CAD build for the part. Positions are in the model's coordinates, mm. A direction names the side the tool comes from. Coordinates: 2 decimals unless noted, no trailing zeros. Write each loop counter-clockwise with the first axis right and the second up, starting at its lowest first coordinate (ties: lowest second). Pieces come first, ordered by that corner, then holes. Notation, with made-up numbers: (49, 49) - (72, 49) arc R28 ccw to (72, 71) - close; hole circle Ø2 at (57.5, 76.25). An arc over 180 degrees is marked (long way). One line per question, with ' | ' between items. Start each with the question number.
1. Band-saw the part on A-A, the plane x = 0. Write the cut outline in (y, z), then the cut area to 4 significant figures.
2. Band-saw the part on C-C, the plane y = 19.5. Write the cut outline in (x, z).
3. Which spindle directions (+Z, -Z, +X, -X, +Y, -Y) get a long thin tool onto all of the face, cutting with end or side? Do faces 1 (the cylindrical face through (0.33, 29.684, -7.493)), 2 (the flat face through (-5, 25, 2)). Say none if no direction does.
4. Flat gauge pins, fed straight in: P1, Ø5, axis at y = -8, z = 0.5, coming from the -X side; P2, Ø4, axis at x = 0, y = 20, coming from the -Z side; P3, Ø3, axis at x = 1.5, y = -9.5, coming from the +Z side. Where does each tip first touch, or does it go through?
5. Band-saw the part on B-B, the plane z = 0. Write the cut outline in (x, y), then the cut area to 4 significant figures.
6. Probe line 1 (X direction, y = -16.5, z = 0.25); line 2 (Y direction, x = 6.25, z = -2); line 3 (X direction, y = 32.5, z = -1.25). List the from-to ranges inside material, lowest first.
from build123d import *

# Parameters (mm, degrees)
SKETCH_1_R      = 5
EXTRUDE_1_DEPTH = 25
SKETCH_2_R      = 7.5
EXTRUDE_2_DEPTH = 10
CHAMFER_1_SIZE  = 0.5


with BuildPart() as part:
    # 草图1 → 凸台-拉伸1 (new, symmetric)
    with BuildSketch(Plane(origin=(0, 0, 0), x_dir=(1, 0, 0), z_dir=(0, 1, 0))):
        with Locations(Location((0, 0, 0), (0, 0, 270))):
            Circle(SKETCH_1_R)
    extrude(amount=EXTRUDE_1_DEPTH, both=True)

    # 草图2 → 凸台-拉伸2 (add)
    with BuildSketch(Plane(origin=(0, 25, 0), x_dir=(1, 0, 0), z_dir=(0, 1, 0))):
        with Locations(Location((0, 0, 0), (0, 0, 270))):
            Circle(SKETCH_2_R)
    extrude(amount=EXTRUDE_2_DEPTH)

    # 倒角1
    chamfer_1_edges = [part.edges().sort_by_distance(p)[0] for p in [
        (0, -25, -5),
        (0, 35, -7.5),
    ]]
    chamfer(chamfer_1_edges, length=CHAMFER_1_SIZE)


solid = part.part
Filled in:
1) outline: (-25, -4.5) - (-24.5, -5) - (25, -5) - (25, -7.5) - (34.5, -7.5) - (35, -7) - (35, 7) - (34.5, 7.5) - (25, 7.5) - (25, 5) - (-24.5, 5) - (-25, 4.5) - close | area: 649.5 mm²
2) outline: circle Ø10 at (0, 0)
3) face 1: +Y, -Y | face 2: -Y
4) P1: stops at x = -5 | P2: stops at z = -5 | P3: stops at z = 5
5) outline: (-7.5, 25) - (-5, 25) - (-5, -24.5) - (-4.5, -25) - (4.5, -25) - (5, -24.5) - (5, 25) - (7.5, 25) - (7.5, 34.5) - (7, 35) - (-7, 35) - (-7.5, 34.5) - close | area: 649.5 mm²
6) line 1: x = -4.99 to 4.99 | line 2: y = 25 to 35 | line 3: x = -7.4 to 7.4
